Source: CAD feature listing. Evaluate the final solid. Frame: model axes, mm. A direction names the side the tool comes from. Coordinates: 2 decimals unless noted, no trailing zeros. Write each loop counter-clockwise with the first axis right and the second up, starting at its lowest first coordinate (ties: lowest second). Pieces come first, ordered by that corner, then holes. Notation, with made-up numbers: (36, 13) - (68, 13) arc R4 ccw to (68, 17) - close; hole circle Ø6 at (-30.5, -18.5). An arc over 180 degrees is marked (long way). One line per item, written item: value.
from build123d import *

# Parameters (mm, degrees)
BRACKET_PROFILE_SKETCH_R   = 7
BRACKET_PROFILE_SKETCH_R_2 = 5
BRACKET_BODY_25MM_DEPTH    = 12.5
EDGE_CHAMFER_5MM_SIZE      = 5
SLOT_SKETCH_W              = 27
SLOT_SKETCH_H              = 33
SLOT_CUT_8MM_DEPTH         = 8
CROSS_HOLE_SKETCH_R        = 38
CROSS_HOLE_CUT_DEPTH       = 5.5


with BuildPart() as part:
    # Bracket Profile Sketch → Bracket Body 25mm (new, symmetric)
    with BuildSketch(Plane.XY):
        with BuildLine():
            Line((16, -3.84), (38, -3.84))
            Line((38, -3.84), (38, -28.84))
            Line((38, -28.84), (12, -61.84))
            Line((12, -61.84), (-1, -61.84))
            ThreePointArc((-1, -61.84), (-5.071476538, -55.587008251), (-8.001806768, -48.724793466))
            ThreePointArc((-8.001806768, -48.724793466), (-11.637006424, -43.74209702), (-17.504200585, -41.84))
            Line((-17.504200585, -41.84), (-47, -41.84))
            Line((-47, -41.84), (-47, -8.84))
            Line((-47, -8.84), (-15.198684154, -8.84))
            ThreePointArc((-15.198684154, -8.84), (2.531901809, -19.638400971), (16, -3.84))
        make_face()
        with Locations((-31, -22.84)):
            Circle(BRACKET_PROFILE_SKETCH_R, mode=Mode.SUBTRACT)
        with Locations((26, -18.84)):
            Circle(BRACKET_PROFILE_SKETCH_R_2, mode=Mode.SUBTRACT)
    extrude(amount=BRACKET_BODY_25MM_DEPTH, both=True)

    # Edge Chamfer 5mm
    edge_chamfer_5mm_edges = [part.edges().sort_by_distance(p)[0] for p in [
        (38, -3.84, 0),
        (-47, -41.84, 0),
        (-47, -8.84, 0),
    ]]
    chamfer(edge_chamfer_5mm_edges, length=EDGE_CHAMFER_5MM_SIZE)

    # Slot Sketch → Slot Cut 8mm (cut)
    with BuildSketch(Plane.XY.offset(12.5)):
        with Locations((-33.5, -25.34)):
            Rectangle(SLOT_SKETCH_W, SLOT_SKETCH_H)
    extrude(amount=-SLOT_CUT_8MM_DEPTH, mode=Mode.SUBTRACT)

    # Cross Hole Sketch → Cross Hole Cut (cut, symmetric)
    with BuildSketch(Plane.XY):
        with Locations((38, -3.84)):
            Circle(CROSS_HOLE_SKETCH_R)
    extrude(amount=CROSS_HOLE_CUT_DEPTH, both=True, mode=Mode.SUBTRACT)


solid = part.part
1) Section query B-B on z = 2.5. Output: boundary loops of the cut face in (x, y), then the cut area to 3 significant figures.
Values found:
outline: (-47, -36.84) - (-42, -41.84) - (-17.5, -41.84) arc R10 cw to (-8, -48.72) arc R43.04 ccw to (-1, -61.84) - (12, -61.84) - (28.67, -40.68) arc R38 cw to (3.37, -19.48) arc R16 cw to (-15.2, -8.84) - (-42, -8.84) - (-47, -13.84) - close; hole circle Ø14 at (-31, -22.84)
area: 2,070 mm2
2) Section query C-C on y = -22.84. Output: boundary loops of the cut face in (x, z).
Values found:
outline: (-47, -12.5) - (-38, -12.5) - (-38, 4.5) - (-47, 4.5) - close; (-24, -12.5) - (23, -12.5) - (23, -5.5) - (5.09, -5.5) - (5.09, 5.5) - (23, 5.5) - (23, 12.5) - (-20, 12.5) - (-20, 4.5) - (-24, 4.5) - close; (29, -12.5) - (38, -12.5) - (38, -5.5) - (29, -5.5) - close; (29, 5.5) - (38, 5.5) - (38, 12.5) - (29, 12.5) - close
3) Reachability of faces 4 (the flat face through (-29, -8.84, -3)), 5 (the flat face through (20, -22, -5.5)), 6 (the flat face through (-37, -29, 4.5)) from +Z, -Z, +X, -X, +Y, -Y: full face, straight path, thin tool, end or side. Return the list, or none.
Values found:
face 4: +Z, -Z, -X, +Y
face 5: +X, +Y
face 6: +Z, -X, +Y, -Y
4) Draft query along Y for faces 1 (the cylindrical face through (21.005, -18.62, -9.049)), 2 (the flat face through (20, -22, 5.5)), 3 (the cylindrical face through (-2.78, -19.597, 0.175)). Return one class per face: released by +Y, released by -Y, zero draft, split by the parting line, or undercut.
Values found:
face 1: undercut
face 2: zero draft
face 3: released by +Y
5) Section query D-D on x = 26. Output: boundary loops of the cut face in (y, z).
Values found:
outline: (-44.07, -12.5) - (-23.84, -12.5) - (-23.84, -5.5) - (-39.9, -5.5) - (-39.9, 5.5) - (-23.84, 5.5) - (-23.84, 12.5) - (-44.07, 12.5) - close; (-13.84, -12.5) - (-3.84, -12.5) - (-3.84, -5.5) - (-13.84, -5.5) - close; (-13.84, 5.5) - (-3.84, 5.5) - (-3.84, 12.5) - (-13.84, 12.5) - close
6) Section query A-A on x = -31. Output: boundary loops of the cut face in (y, z).
Values found:
outline: (-41.84, -12.5) - (-29.84, -12.5) - (-29.84, 4.5) - (-41.84, 4.5) - close; (-15.84, -12.5) - (-8.84, -12.5) - (-8.84, 4.5) - (-15.84, 4.5) - close
7) Contact query for flat-ended pins moving along their axis: P1, Ø10, axis at y = -48, z = -6.5, coming from the -X side; P2, Ø4, axis at y = -21, z = 9, coming from the -X side; P3, Ø5, axis at y = -40.5, z = 6.5, coming from the +X side; P4, Ø16, axis at x = 26, y = -18.84, coming from the -Z side. Output: stop coordinate, or through.
Values found:
P1: x = -12.83
P2: x = -20
P3: x = 30.78
P4: z = -12.5
8) Material intervals for line 1 (Z direction, x = 12.5, y = -17.5); line 2 (Y direction, x = -31, z = -5.25); line 3 (Y direction, x = -0.5, z = -5.5), sorted ascending.
Values found:
line 1: -12.5 to -5.5, 5.5 to 12.5
line 2: -41.84 to -29.84, -15.84 to -8.84
line 3: -61.84 to -19.83
